Part model, mm, in its own coordinate system. A direction names the side the tool comes from. Round coordinates to 2 decimals unless told otherwise and drop trailing zeros. Write each loop counter-clockwise with the first axis right and the second up, starting at its lowest first coordinate (ties: lowest second). Pieces come first, ordered by that corner, then holes.
```python
from build123d import *

# Parameters (mm, degrees)
SKETCH1_R           = 9
BOSS_EXTRUDE1_DEPTH = 37.5
SKETCH2_R           = 10
BOSS_EXTRUDE2_DEPTH = 21.5
CHAMFER1_SIZE       = 0.5


with BuildPart() as part:
    # Sketch1 → Boss-Extrude1 (new body)
    with BuildSketch(Plane.XY):
        Circle(SKETCH1_R)
    extrude(amount=BOSS_EXTRUDE1_DEPTH)

    # Sketch2 → Boss-Extrude2 (add)
    with BuildSketch(Plane(origin=(0, 0, 0), x_dir=(-1, 0, 0), z_dir=(0, 0, -1))):
        Circle(SKETCH2_R)
    extrude(amount=-BOSS_EXTRUDE2_DEPTH)

    # Chamfer1
    chamfer1_edges = [part.edges().sort_by_distance(p)[0] for p in [
        (-9, 0, 37.5),
        (10, 0, 21.5),
        (10, 0, 0),
    ]]
    chamfer(chamfer1_edges, length=CHAMFER1_SIZE)


solid = part.part
```
Q1. Which spindle directions (+Z, -Z, +X, -X, +Y, -Y) get a long thin tool onto all of the face, cutting with end or side? Do faces 3 (the cylindrical face through (-1.172, 8.923, 29.142)), 4 (the flat face through (0, 0, 0)). Say none if no direction does.
Values follow:
face 3: +Z
face 4: -Z, +X, -X, +Y, -Y
Q2. Mould opens along Y. For faces 1 (the flat face through (6, -7, 21.5)), 2 (the cylindrical face through (2.17, -9.76, 10.61)) say: +Y half, -Y half, draft (parallel to the pull), parting line (faces both ways), or undercut.
Values follow:
face 1: draft
face 2: parting line
Q3. Cut at A-A on y = 0. Write the cut outline in (x, z).
Values follow:
outline: (-10, 0.5) - (-9.5, 0) - (9.5, 0) - (10, 0.5) - (10, 21) - (9.5, 21.5) - (9, 21.5) - (9, 37) - (8.5, 37.5) - (-8.5, 37.5) - (-9, 37) - (-9, 21.5) - (-9.5, 21.5) - (-10, 21) - close
Q4. Cut at C-C on z = 7.5. Write the cut outline in (x, y), plus the area to 3 significant figures.
Values follow:
outline: circle Ø20 at (0, 0)
area: 314 mm2
Q5. Drop flat-ended pins along their axis: pin 1 (3 mm diameter, centred on x = 3.5, z = 29.5, fed in from +Y); pin 2 (12 mm diameter, centred on x = 6.5, z = 32.5, fed in from -Y); pin 3 (12 mm diameter, centred on y = 6.5, z = 19, fed in from +X). Give the stop position or say it passes through.
Values follow:
pin 1: stops at y = 8.77
pin 2: stops at y = -8.99
pin 3: stops at x = 9.99
Q6. Wall check: L1, parallel to Z at x = 3.75, y = -8.25; L2, parallel to X at y = -4.5, z = 5; L3, parallel to X at y = 5.5, z = 24.5. Give the ranges that are in metal, low to high.
Values follow:
L1: z = 0 to 21.5
L2: x = -8.93 to 8.93
L3: x = -7.12 to 7.12
